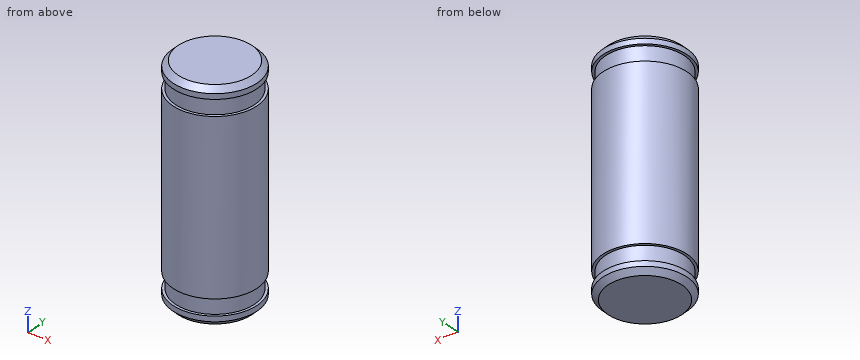
from build123d import *

# Parameters (mm, degrees)
SKETCH1_R                = 4
BOSS_EXTRUDE1_DEPTH      = 8
SKETCH2_R                = 3.75
BOSS_EXTRUDE2_DEPTH      = 1.5
BOSS_EXTRUDE3_START      = 1
SKETCH3_R                = 4
BOSS_EXTRUDE3_DEPTH      = 1
CHAMFER1_SIZE            = 0.5
CHAMFER1_OF_MIRROR1_SIZE = 0.5


with BuildPart() as part:
    # Sketch1 → Boss-Extrude1 (new, symmetric)
    with BuildSketch(Plane.XY):
        Circle(SKETCH1_R)
    extrude(amount=BOSS_EXTRUDE1_DEPTH, both=True)

    # Sketch2 → Boss-Extrude2 (add)
    with BuildSketch(Plane.XY.offset(8)):
        Circle(SKETCH2_R)
    boss_extrude2 = extrude(amount=BOSS_EXTRUDE2_DEPTH)

    # Sketch3 → Boss-Extrude3 (add)
    with BuildSketch(Plane.XY.offset(9.5).offset(BOSS_EXTRUDE3_START)):
        Circle(SKETCH3_R)
    boss_extrude3 = extrude(amount=-BOSS_EXTRUDE3_DEPTH)

    # Chamfer1
    chamfer1_edges = [part.edges().sort_by_distance(p)[0] for p in [
        (-4, 0, 10.5),
    ]]
    chamfer(chamfer1_edges, length=CHAMFER1_SIZE)

    # Mirror1: Boss-Extrude2, Boss-Extrude3 across plane
    add(boss_extrude2.mirror(Plane.XY))
    add(boss_extrude3.mirror(Plane.XY))

    # Chamfer1 of Mirror1
    chamfer1_of_mirror1_edges = [part.edges().sort_by_distance(p)[0] for p in [
        (-4, 0, -10.5),
    ]]
    chamfer(chamfer1_of_mirror1_edges, length=CHAMFER1_OF_MIRROR1_SIZE)


solid = part.part
Build history of the part. All positions in model axes, mm. Round coordinates to 2 decimals unless told otherwise and drop trailing zeros. Write each loop counter-clockwise with the first axis right and the second up, starting at its lowest first coordinate (ties: lowest second). Pieces come first, ordered by that corner, then holes. Notation, with made-up numbers: (-11.75, 1) -> (25.25, 1) arc R35 ccw to (25.25, 39) -> close; hole circle Ø11 at (53.5, -23). An arc over 180 degrees is marked (long way). Use one line per item in the form item = value.
Q1. Drill centre lines: L1, parallel to Z at x = -2, y = -3.25; L2, parallel to Y at x = -1.5, z = -1.25; L3, parallel to Y at x = -2.25, z = 2.75. Where is each one in solid material? Low to high.
Conclusion:
L1 = -10.18 to -9.5, -8 to 8, 9.5 to 10.18
L2 = -3.71 to 3.71
L3 = -3.31 to 3.31
Q2. Drop flat-ended pins along their axis: P1, Ø3, axis at x = -3, y = -2, coming from the -Z side; P2, Ø2, axis at y = -1.5, z = -5.5, coming from the -X side. Give the stop position or say it passes through.
Conclusion:
P1 = -10.5
P2 = -3.97
Q3. Band-saw the part on A-A, the plane z = -4.5. Write the cut outline in (x, y).
Conclusion:
outline = circle Ø8 at (0, 0)
Q4. Band-saw the part on B-B, the plane z = 8.5. Write the cut outline in (x, y).
Conclusion:
outline = circle Ø7.5 at (0, 0)
